from build123d import *

# Parameters (mm, degrees)
CUT_EXTRUDE1_DEPTH      = 1.2
CUT_EXTRUDE1_DEPTH_BACK = 1.2
SKETCH3_W               = 11
SKETCH3_H               = 11


with BuildPart() as part:
    # Sketch1 → Revolve1 (revolve)
    with BuildSketch(Plane.XY, mode=Mode.PRIVATE) as revolve1_sk:
        with BuildLine():
            Line((-1.2, 0), (-1.2, 2.76))
            ThreePointArc((-1.2, 2.76), (-1.041837662, 3.141837662), (-0.66, 3.3))
            Line((-0.66, 3.3), (1.2, 3.3))
            Line((1.2, 3.3), (1.2, 0))
            Line((1.2, 0), (-1.2, 0))
        make_face()
    revolve(revolve1_sk.sketch.rotate(Axis((1.2, 0, 0), (-1, 0, 0)), 270), axis=Axis((1.2, 0, 0), (-1, 0, 0)))

    # Sketch2 → Cut-Revolve1 (revolve, cut)
    with BuildSketch(Plane.XY, mode=Mode.PRIVATE) as cut_revolve1_sk:
        Polygon((-1.2, 0), (-1.2, 1.5), (-0.9295, 1.2295), (0.9295, 1.2295), (1.2, 1.5), (1.2, 0), align=None)
    revolve(cut_revolve1_sk.sketch.rotate(Axis((1.2, 0, 0), (-1, 0, 0)), 270), axis=Axis((1.2, 0, 0), (-1, 0, 0)), mode=Mode.SUBTRACT)

    # Sketch3 → Cut-Extrude1 (cut, two sides: drawn at the far end of the back side and taken through both)
    with BuildSketch(Plane(origin=(0, 0, 0), x_dir=(0, 0, -1), z_dir=(1, 0, 0)).offset(-CUT_EXTRUDE1_DEPTH_BACK)):
        Rectangle(SKETCH3_W, SKETCH3_H)
        Polygon((-2.75, 1.58771324), (-2.75, -1.58771324), (0, -3.175426481), (2.75, -1.58771324), (2.75, 1.58771324), (0, 3.175426481), align=None, mode=Mode.SUBTRACT)
    extrude(amount=CUT_EXTRUDE1_DEPTH + CUT_EXTRUDE1_DEPTH_BACK, mode=Mode.SUBTRACT)


solid = part.part
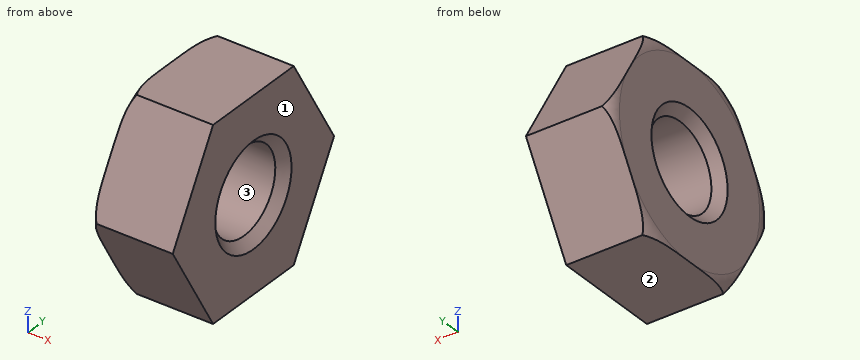
For this review, take the finished solid that the model builds, in its own axes (mm). Face numbers are marked on the shaded views. Round coordinates to 2 decimals unless told otherwise and drop trailing zeros. Loops run counter-clockwise (first coordinate to the right, second up) from the corner with the lowest first, then second, coordinate; pieces in that order, holes last. Notation, with made-up numbers: (-21, 1) - (10, 1) arc R4 cw to (10, 7) - close; hole circle Ø4 at (59, -34.5). An arc over 180 degrees is marked (long way). One line per item, written item: value. Start each with the question number.
Item 1: For L1, parallel to Z at x = 0.5, y = 0.5; L2, parallel to Y at x = 0.55, z = 1.05; L3, parallel to Y at x = 0.2, z = -0.45, list the stretches that pass through material, from the lowest coordinate up.
Item 2: The part is to be moulded in two halves that separate along Z. For the marked faces 1, 2 and 3, say which applies: +Z half, -Z half, draft (parallel to the pull), parting line (faces both ways), or undercut.
Item 3: Take a section at C-C (x = -0.3). Give the boundary of the cut face in (y, z), plus the area to 3 significant figures.
Item 4: Take a section at A-A (x = 1). Give the boundary of the cut face in (y, z), plus the area to 3 significant figures.
Item 5: Take a section at B-B (y = 0). Give the boundary of the cut face in (x, z), plus the area to 3 significant figures.
Item 6: Clearance check with a flat-ended pin moving along its axis: pin 1 Ø1.5 at (y, z) = (0, 0) entering from +X. State where the tip first meets the part, or that it passes through.
Answer below:
1. L1: z = -2.75 to -1.12, 1.12 to 2.75
1. L2: y = -2.57 to -0.64, 0.64 to 2.57
1. L3: y = -2.92 to -1.14, 1.14 to 2.92
2. face 1: draft
2. face 2: -Z half
2. face 3: undercut
3. outline: (-3.18, 0) - (-1.59, -2.75) - (1.59, -2.75) - (3.18, 0) - (1.59, 2.75) - (-1.59, 2.75) - close; hole circle Ø2.46 at (0, 0)
3. area: 21.4 mm2
4. outline: (-3.18, 0) - (-1.59, -2.75) - (1.59, -2.75) - (3.18, 0) - (1.59, 2.75) - (-1.59, 2.75) - close; hole circle Ø2.6 at (0, 0)
4. area: 20.9 mm2
5. outline: (-1.2, -2.75) - (1.2, -2.75) - (1.2, -1.5) - (0.93, -1.23) - (-0.93, -1.23) - (-1.2, -1.5) - close; (-1.2, 1.5) - (-0.93, 1.23) - (0.93, 1.23) - (1.2, 1.5) - (1.2, 2.75) - (-1.2, 2.75) - close
5. area: 7.15 mm2
6. pin 1: passes through
